Build history of the part. All positions in model axes, mm. A direction names the side the tool comes from. Give positions to 0.01 mm unless a question says otherwise; leave off trailing zeros. Loops run counter-clockwise (first coordinate to the right, second up) from the corner with the lowest first, then second, coordinate; pieces in that order, holes last. Notation, with made-up numbers: (89.5, 75) - (113.5, 75) arc R17 ccw to (113.5, 102) - close; hole circle Ø1 at (10.5, -0.5). An arc over 180 degrees is marked (long way). Return JSON: item names as keys, results as strings. Group by question number.
1) Drop flat-ended pins along their axis: pin 1 (3 mm diameter, centred on x = 34, z = -2, fed in from -Y); pin 2 (4 mm diameter, centred on x = 63.5, y = -9, fed in from -Z); pin 3 (2 mm diameter, centred on x = 79.5, z = -9.5, fed in from +Y); pin 4 (10 mm diameter, centred on x = 85.5, y = -0.5, fed in from +Z). Give the stop position or say it passes through.
2) Drill centre lines: probe 1 along X at (y, z) = (8, 7); probe 2 along Z at (x, y) = (52, -4.25); probe 3 along Y at (x, z) = (104, -5) (3 decimals). Where is each one in solid material? Low to high. Write a range as from..to.
3) Slice it at B-B (x = 7). List the corners of the cut face in (y, z), and give its area (3 significant figures).
4) 3-axis set-ups, long thin cutter, end or side, ignore diameter. For faces 1 (the face through (4.93, 10.44, 5.92)), 2 (the face through (60.91, 7.81, -1.73)): which of +Z, -Z, +X, -X, +Y, -Y reach the whole face in a straight line?
5) Slice it at A-A (x = 85). List the corners of the cut face in (y, z).
```python
from build123d import *

# Parameters (mm, degrees)
BOSS_EXTRUDE1_DEPTH = 10
SKETCH4_R           = 26.17
SKETCH4_R_2         = 12
CUT_EXTRUDE1_DEPTH  = 1.25
CUT_EXTRUDE1_DRAFT  = -60
CHAMFER2_SIZE       = 0.888888889


with BuildPart() as part:
    # Sketch3 → Boss-Extrude1 (new body)
    with BuildSketch(Plane(origin=(0, 0, 0), x_dir=(0, 0, -1), z_dir=(1, 0, 0))):
        Polygon((12, 6.92820323), (0, 13.856406461), (-12, 6.92820323), (-12, -6.92820323), (0, -13.856406461), (12, -6.92820323), align=None)
    extrude(amount=BOSS_EXTRUDE1_DEPTH)


with BuildPart() as cut_extrude1_tool:
    # Sketch4 → Cut-Extrude1 (with draft: the straight prism first)
    with BuildSketch(Plane.ZY):
        Circle(SKETCH4_R)
        Circle(SKETCH4_R_2, mode=Mode.SUBTRACT)
    extrude(amount=-CUT_EXTRUDE1_DEPTH)
    # Cut-Extrude1: the draft: its side faces are tilted about the plane it starts from
    cut_extrude1_sides = [cut_extrude1_tool.faces().sort_by_distance(p)[0] for p in [
        (0.625, 0, -26.17),
        (0.625, 0, -12),
    ]]
    draft(cut_extrude1_sides, Plane.ZY, CUT_EXTRUDE1_DRAFT)


with BuildPart() as part_1:
    add(part.part)

    # Cut-Extrude1: cut by cut_extrude1_tool
    add(cut_extrude1_tool.part, mode=Mode.SUBTRACT)

    # Sketch5 → Revolve1 (revolve)
    with BuildSketch(Plane.XY, mode=Mode.PRIVATE) as revolve1_sk:
        with BuildLine():
            Line((11.35, 8), (110, 8))
            Line((110, 8), (110, 0))
            Line((110, 0), (10, 0))
            Line((10, 0), (10, 9.35))
            ThreePointArc((10, 9.35), (10.395405845, 8.395405845), (11.35, 8))
        make_face()
    revolve(revolve1_sk.sketch.rotate(Axis((10, 0, 0), (1, 0, 0)), 90), axis=Axis((10, 0, 0), (1, 0, 0)))

    # Chamfer2
    chamfer2_edges = [part_1.edges().sort_by_distance(p)[0] for p in [
        (110, 0, -8),
    ]]
    chamfer(chamfer2_edges, length=CHAMFER2_SIZE)


solid = part_1.part
```
Results:
{
 "1": {"pin 1": "y = -7.98", "pin 2": "z = -3.87", "pin 3": "through", "pin 4": "z = 8"},
 "2": {"probe 1": "0..10", "probe 2": "-6.78..6.78", "probe 3": "-6.245..6.245"},
 "3": {"outline": "(-13.86, 0) - (-6.93, -12) - (6.93, -12) - (13.86, 0) - (6.93, 12) - (-6.93, 12) - close", "area": "499 mm2"},
 "4": {"face 1": "+Z, +X, -X, +Y", "face 2": "+X"},
 "5": {"outline": "circle Ø16 at (0, 0)"}
}
